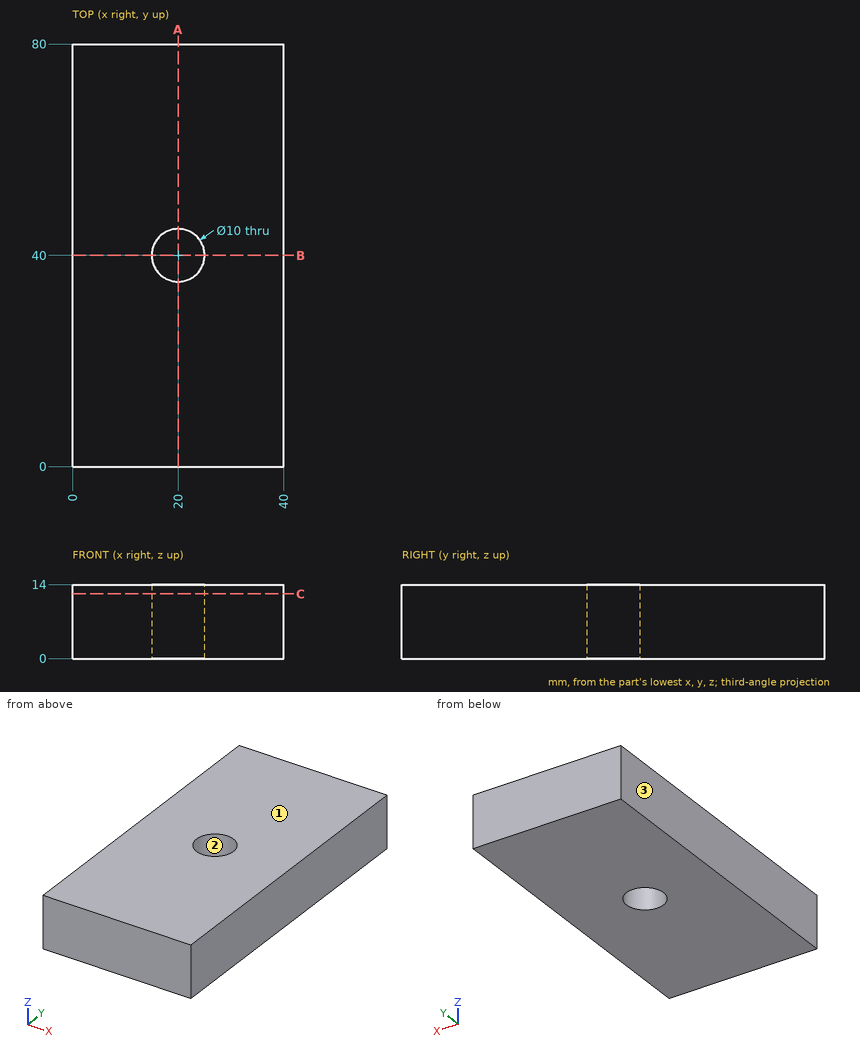
Geometry: see drawing. Coordinates: mm, zero at the bounding-box minimum. Give positions to 0.01 mm unless a question says otherwise; leave off trailing zeros. Order: outer loops, then holes, each group sorted by start corner. A loop starts at its lowest first (then second) coordinate and runs counter-clockwise, first axis right, second up.
1. Cut plane A-A (x = 20). Return loops of the section in (y, z), and give its area (3 significant figures).
Computed:
outline: (0, 0) - (35, 0) - (35, 14) - (0, 14) - close; (45, 0) - (80, 0) - (80, 14) - (45, 14) - close
area: 980 mm2
2. Cut plane B-B (y = 40). Return loops of the section in (x, z).
Computed:
outline: (0, 0) - (15, 0) - (15, 14) - (0, 14) - close; (25, 0) - (40, 0) - (40, 14) - (25, 14) - close
3. Cut plane C-C (z = 12.25). Return loops of the section in (x, y), and give its area (3 significant figures).
Computed:
outline: (0, 0) - (40, 0) - (40, 80) - (0, 80) - close; hole circle Ø10 at (20, 40)
area: 3,120 mm2
4. Draft query along X for the marked faces 1, 2 and 3. Return one class per face: released by +X, released by -X, zero draft, split by the parting line, or undercut.
Computed:
face 1: zero draft
face 2: undercut
face 3: released by -X
5. Line query: probe 1 along Y at (x, z) = (20, 4.5); probe 2 along Y at (x, z) = (17.5, 8.25); probe 3 along X at (y, z) = (38, 8.5). Output: solid intervals per line, ascending.
Computed:
probe 1: y = 0 to 35, 45 to 80
probe 2: y = 0 to 35.67, 44.33 to 80
probe 3: x = 0 to 15.42, 24.58 to 40
